Read the model definition and answer for the solid it produces. Units are mm, in the model's axes. A direction names the side the tool comes from. Give positions to 0.01 mm unless a question says otherwise; leave off trailing zeros. Order: outer loops, then holes, each group sorted by start corner. A loop starts at its lowest first (then second) coordinate and runs counter-clockwise, first axis right, second up.
```python
from build123d import *

# Parameters (mm, degrees)
SKETCH2_R          = 11.5
CUT_EXTRUDE1_DEPTH = 1
SKETCH3_R          = 10
CUT_EXTRUDE2_DEPTH = 1.25
SKETCH4_R          = 2.5
CUT_EXTRUDE3_DEPTH = 8.5


with BuildPart() as part:
    # Sketch1 → Revolve1 (revolve)
    with BuildSketch(Plane.XY, mode=Mode.PRIVATE) as revolve1_sk:
        with BuildLine():
            Line((0, 0), (5, 0))
            Line((5, 0), (5, 12.5))
            Line((5, 12.5), (3, 12.5))
            Line((3, 12.5), (3, 12))
            ThreePointArc((3, 12), (2.707106781, 11.292893219), (2, 11))
            Line((2, 11), (0, 11))
            Line((0, 11), (0, 0))
        make_face()
    revolve1 = revolve(revolve1_sk.sketch.rotate(Axis((0, 0, 0), (1, 0, 0)), 90), axis=Axis((0, 0, 0), (1, 0, 0)))

    # Mirror1: Revolve1 across plane
    add(revolve1.mirror(Plane(origin=(0, 0, 0), x_dir=(0, 0, 1), z_dir=(1, 0, 0))))

    # Sketch2 → Cut-Extrude1 (cut)
    with BuildSketch(Plane(origin=(5, 0, 0), x_dir=(0, 0, -1), z_dir=(1, 0, 0))):
        Circle(SKETCH2_R)
    cut_extrude1 = extrude(amount=-CUT_EXTRUDE1_DEPTH, mode=Mode.SUBTRACT)

    # Sketch3 → Cut-Extrude2 (cut)
    with BuildSketch(Plane(origin=(4, 0, 0), x_dir=(0, 0, -1), z_dir=(1, 0, 0))):
        Circle(SKETCH3_R)
    cut_extrude2 = extrude(amount=-CUT_EXTRUDE2_DEPTH, mode=Mode.SUBTRACT)

    # Mirror3: Cut-Extrude1, Cut-Extrude2 across plane
    add(cut_extrude1.mirror(Plane(origin=(0, 0, 0), x_dir=(0, 0, 1), z_dir=(1, 0, 0))), mode=Mode.SUBTRACT)
    add(cut_extrude2.mirror(Plane(origin=(0, 0, 0), x_dir=(0, 0, 1), z_dir=(1, 0, 0))), mode=Mode.SUBTRACT)

    # Sketch4 → Cut-Extrude3 (cut)
    with BuildSketch(Plane(origin=(2.75, 0, 0), x_dir=(0, 0, -1), z_dir=(1, 0, 0))):
        with Locations((0, 7)):
            Circle(SKETCH4_R)
        with Locations((7, 0)):
            Circle(SKETCH4_R)
        with Locations((0, -7)):
            Circle(SKETCH4_R)
        with Locations((-7, 0)):
            Circle(SKETCH4_R)
        Circle(SKETCH4_R)
    extrude(amount=-CUT_EXTRUDE3_DEPTH, mode=Mode.SUBTRACT)


solid = part.part
```
1) The part is cut by section C-C on x = -4.5. Determine the outline of the cut face in (y, z).
Final values:
outline: circle Ø25 at (0, 0); hole circle Ø23 at (0, 0)
2) Consider L1, parallel to Y at x = -1.1, z = 0; L2, parallel to Y at x = 3.65, z = 0; L3, parallel to X at y = 9.5, z = -8. Determine where each line is inside the solid, lowest interval first.
Final values:
L1: y = -11 to -9.5, -4.5 to -2.5, 2.5 to 4.5, 9.5 to 11
L2: y = -12.5 to -10, 10 to 12.5
L3: x = -5 to -3, 3 to 5
3) The part is cut by section D-D on x = -1.5. Determine the outline of the cut face in (y, z), and give its area (3 significant figures).
Final values:
outline: circle Ø22 at (0, 0); hole circle Ø5 at (-7, 0); hole circle Ø5 at (0, -7); hole circle Ø5 at (0, 0); hole circle Ø5 at (0, 7); hole circle Ø5 at (7, 0)
area: 282 mm2
4) The part is cut by section A-A on z = 0. Count the separate pieces of the cut face and the enclosed holes in it, and give its area (3 significant figures).
Final values:
separate pieces: 4
enclosed holes: 0
area: 54.4 mm2
5) For a pull along Z with two mould halves and no side action, classify faces 1 (the face through (-3, -10, -7)), 2 (the face through (0.038, 0.751, 4.615)), 3 (the face through (-3.986, -3.755, 11.923)) as released by +Z, released by -Z, zero draft, split by the parting line, or undercut.
Final values:
face 1: zero draft
face 2: undercut
face 3: split by the parting line
6) A tool of negligible diameter and unlimited length cuts with its end or side. For faces 4 (the face through (3.38, -9.76, 2.17)), 5 (the face through (-2.75, -2, -2)), 6 (the face through (3, -10, -7)), from which of +Z, -Z, +X, -X, +Y, -Y can it reach the whole face along a straight path? Write none if from no direction.
Final values:
face 4: +X
face 5: -X
face 6: none
7) Given pin 1 (7.5 mm diameter, centred on y = -0.5, z = -2, fed in from -X); pin 2 (5 mm diameter, centred on y = 1, z = -7.5, fed in from -X); pin 3 (4 mm diameter, centred on y = -9.5, z = 8.5, fed in from -X); pin 4 (6 mm diameter, centred on x = 1, z = -4, fed in from -Y), each flat-ended and moving along its own axis, determine where each tip first touches the part or whether it passes through.
Final values:
pin 1: stops at x = -2.75
pin 2: stops at x = -4
pin 3: stops at x = -5
pin 4: stops at y = -12.37
